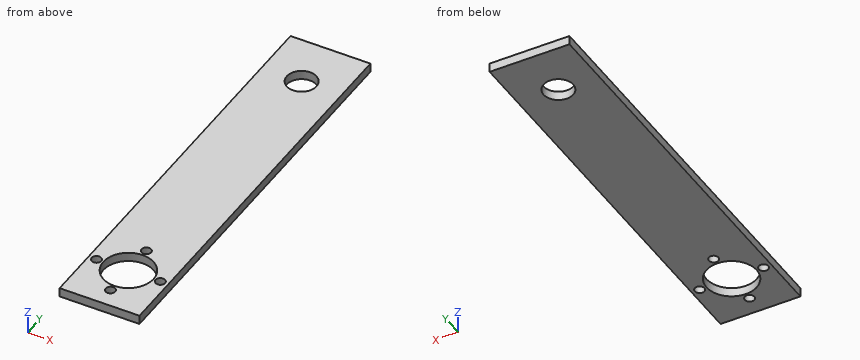
from build123d import *

# Parameters (mm, degrees)
SKETCH1_W           = 35
SKETCH1_H           = 180
SKETCH1_R           = 6.5
SKETCH1_R_2         = 11
BOSS_EXTRUDE1_DEPTH = 4
SKETCH2_R           = 2.1
CUT_EXTRUDE2_DEPTH  = 10


with BuildPart() as part:
    # Sketch1 → Boss-Extrude1 (new body)
    with BuildSketch(Plane.XY):
        with Locations((17.5, -90)):
            Rectangle(SKETCH1_W, SKETCH1_H)
        with Locations((17.5, -22.5)):
            Circle(SKETCH1_R, mode=Mode.SUBTRACT)
        with Locations((17.5, -157.5)):
            Circle(SKETCH1_R_2, mode=Mode.SUBTRACT)
    extrude(amount=BOSS_EXTRUDE1_DEPTH)

    # Sketch2 → Cut-Extrude2 (cut)
    with BuildSketch(Plane.XY.offset(4)):
        with Locations((3.5, -157.5)):
            Circle(SKETCH2_R)
        with Locations((17.5, -143.5)):
            Circle(SKETCH2_R)
        with Locations((31.5, -157.5)):
            Circle(SKETCH2_R)
        with Locations((17.5, -171.5)):
            Circle(SKETCH2_R)
    extrude(amount=-CUT_EXTRUDE2_DEPTH, mode=Mode.SUBTRACT)


solid = part.part
The model under review builds one solid part; all positions refer to its coordinate system, in mm. Round coordinates to 2 decimals unless told otherwise and drop trailing zeros. Order: outer loops, then holes, each group sorted by start corner. A loop starts at its lowest first (then second) coordinate and runs counter-clockwise, first axis right, second up. Notation, with made-up numbers: (49, 55) -> (103, 55) arc R18 ccw to (103, 61) -> close; hole circle Ø9 at (3.25, 48). An arc over 180 degrees is marked (long way). Write item = value, one per line. Start each with the question number.
Item 1: Consider section A-A on y = -157.5. Write out the cut boundary in (x, z).
Item 2: Consider section C-C on z = 2.9. Write out the cut boundary in (x, y).
Item 3: Consider section D-D on y = -22.5. Write out the cut boundary in (x, z).
Item 4: For line 1 along Y through (x, z) = (17.5, 0.9); line 2 along Y through (x, z) = (3.5, 3.25); line 3 along Y through (x, z) = (14, 1.15), list the stretches that pass through material, from the lowest coordinate up.
Item 5: Consider section B-B on x = 31.5. Write out the cut boundary in (y, z), plus the area to 3 significant figures.
Conclusion:
q1.outline = (0, 0) -> (1.4, 0) -> (1.4, 4) -> (0, 4) -> close; (5.6, 0) -> (6.5, 0) -> (6.5, 4) -> (5.6, 4) -> close; (28.5, 0) -> (29.4, 0) -> (29.4, 4) -> (28.5, 4) -> close; (33.6, 0) -> (35, 0) -> (35, 4) -> (33.6, 4) -> close
q2.outline = (0, -180) -> (35, -180) -> (35, 0) -> (0, 0) -> close; hole circle Ø4.2 at (3.5, -157.5); hole circle Ø22 at (17.5, -157.5); hole circle Ø13 at (17.5, -22.5); hole circle Ø4.2 at (17.5, -171.5); hole circle Ø4.2 at (17.5, -143.5); hole circle Ø4.2 at (31.5, -157.5)
q3.outline = (0, 0) -> (11, 0) -> (11, 4) -> (0, 4) -> close; (24, 0) -> (35, 0) -> (35, 4) -> (24, 4) -> close
q4.line_1 = -180 to -173.6, -169.4 to -168.5, -146.5 to -145.6, -141.4 to -29, -16 to 0
q4.line_2 = -180 to -159.6, -155.4 to 0
q4.line_3 = -180 to -167.93, -147.07 to -27.98, -17.02 to 0
q5.outline = (-180, 0) -> (-159.6, 0) -> (-159.6, 4) -> (-180, 4) -> close; (-155.4, 0) -> (0, 0) -> (0, 4) -> (-155.4, 4) -> close
q5.area = 703 mm2
